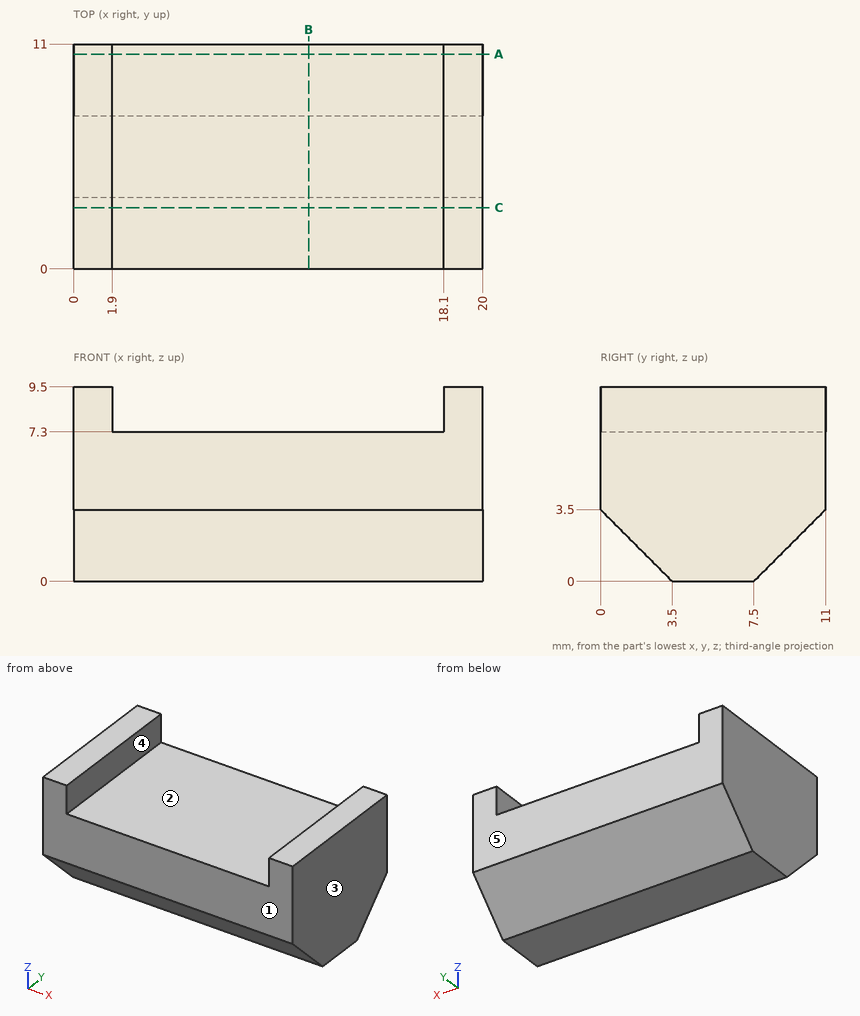
Can you work these out from the drawing? Everything is in mm from the part's minimum corner. A direction names the side the tool comes from. Coordinates: 2 decimals unless noted, no trailing zeros. Order: outer loops, then holes, each group sorted by start corner. A loop starts at its lowest first (then second) coordinate and runs counter-clockwise, first axis right, second up. Notation, with made-up numbers: (43.25, -13.75) -> (76.25, -13.75) arc R32 ccw to (76.25, 20.25) -> close; hole circle Ø4 at (13.5, 67.25). An arc over 180 degrees is marked (long way). Use one line per item in the form item = value.
Q1. Will these pins go through, and if not, where does the flat tip stop? P1, Ø1.5, axis at x = 11.5, z = 1.5, coming from the +Y side; P2, Ø3, axis at x = 8.5, y = 8.5, coming from the +Z side.
From the geometry:
P1 = 9.75
P2 = 7.3
Q2. Imagine slicing it at B-B, the plane x = 11.5. List the corners of the cut face in (y, z) for me.
From the geometry:
outline = (0, 3.5) -> (3.5, 0) -> (7.5, 0) -> (11, 3.5) -> (11, 7.3) -> (0, 7.3) -> close
Q3. Imagine slicing it at C-C, the plane y = 3. List the corners of the cut face in (x, z) for me.
From the geometry:
outline = (0, 0.5) -> (20, 0.5) -> (20, 9.5) -> (18.1, 9.5) -> (18.1, 7.3) -> (1.9, 7.3) -> (1.9, 9.5) -> (0, 9.5) -> close
Q4. Which directions (+Z, -Z, +X, -X, +Y, -Y) give clear straight access to the entire face, cutting with the end or side of a thin tool? Please do the marked faces 1 and 2.
From the geometry:
face_1 = +Z, -Z, +X, -X, -Y
face_2 = +Z, +Y, -Y
Q5. We'd pull the mould along X, two halves only. Please class the marked faces 3, 4 and 5: released by +X, released by -X, zero draft, split by the parting line, or undercut.
From the geometry:
face_3 = released by +X
face_4 = undercut
face_5 = zero draft
Q6. Imagine slicing it at A-A, the plane y = 10.5. List the corners of the cut face in (x, z) for me.
From the geometry:
outline = (0, 3) -> (20, 3) -> (20, 9.5) -> (18.1, 9.5) -> (18.1, 7.3) -> (1.9, 7.3) -> (1.9, 9.5) -> (0, 9.5) -> close
Q7. I need wall thicknesses on L1, parallel to X at y = 8.5, z = 8; L2, parallel to Z at x = 17.5, y = 7.25; L3, parallel to Y at x = 18.5, z = 2. Which ranges of each line are inside material? Lowest first, please.
From the geometry:
L1 = 0 to 1.9, 18.1 to 20
L2 = 0 to 7.3
L3 = 1.5 to 9.5
